Check sheet for the drawn part. Datum: minimum x, y, z corner. Units: mm. A direction names the side the tool comes from. Round coordinates to 2 decimals unless told otherwise and drop trailing zeros. Loops run counter-clockwise (first coordinate to the right, second up) from the corner with the lowest first, then second, coordinate; pieces in that order, holes last.
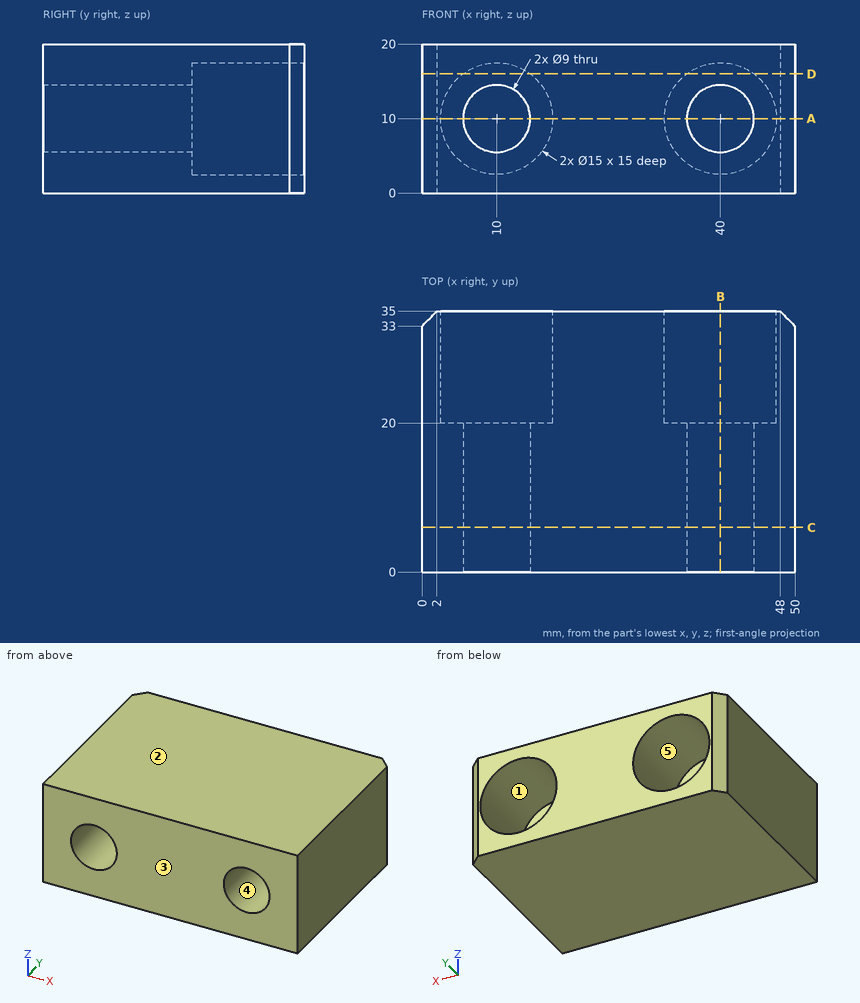
1. Release check for a two-part mould opening along Z. For the marked faces 1, 2 and 3 record: released by +Z, released by -Z, zero draft, split by the parting line, or undercut.
2. Section check D-D (z = 16). Enter the section's corners in (x, y).
3. Section check A-A (z = 10). Enter the section's corners in (x, y).
4. Scan lines: L1, parallel to Z at x = 10, y = 27; L2, parallel to X at y = 27, z = 7; L3, parallel to X at y = 18.5, z = 6.5. Record each from-to range of solid material in increasing order.
5. Gauge pin test, flat ends, axial feed: P1, Ø7.5, axis at x = 39.5, z = 13.5, coming from the +Y side; P2, Ø8, axis at x = 40, z = 10, coming from the -Y side. Record the tip position at first contact, or that the pin passes through.
6. Tool access check on the marked faces 4 and 5. Record the directions out of +Z, -Z, +X, -X, +Y, -Y that give a thin tool (end or side, any length) a straight path to the whole face; none if there is none.
7. Section check B-B (x = 40). Enter the section's corners in (y, z), then the cut area to 3 significant figures.
8. Section check C-C (y = 6). Enter the section's corners in (x, z), then the cut area to 3 significant figures.
Taken from the geometry:
1. face 1: undercut
1. face 2: released by +Z
1. face 3: zero draft
2. outline: (0, 0) - (50, 0) - (50, 33) - (48, 35) - (44.5, 35) - (44.5, 20) - (35.5, 20) - (35.5, 35) - (14.5, 35) - (14.5, 20) - (5.5, 20) - (5.5, 35) - (2, 35) - (0, 33) - close
3. outline: (0, 0) - (5.5, 0) - (5.5, 20) - (2.5, 20) - (2.5, 35) - (2, 35) - (0, 33) - close; (14.5, 0) - (35.5, 0) - (35.5, 20) - (32.5, 20) - (32.5, 35) - (17.5, 35) - (17.5, 20) - (14.5, 20) - close; (44.5, 0) - (50, 0) - (50, 33) - (48, 35) - (47.5, 35) - (47.5, 20) - (44.5, 20) - close
4. L1: z = 0 to 2.5, 17.5 to 20
4. L2: x = 0 to 3.13, 16.87 to 33.13, 46.87 to 50
4. L3: x = 0 to 7.17, 12.83 to 37.17, 42.83 to 50
5. P1: stops at y = 20
5. P2: passes through
6. face 4: +Y, -Y
6. face 5: +Y
7. outline: (0, 0) - (35, 0) - (35, 2.5) - (20, 2.5) - (20, 5.5) - (0, 5.5) - close; (0, 14.5) - (20, 14.5) - (20, 17.5) - (35, 17.5) - (35, 20) - (0, 20) - close
7. area: 295 mm2
8. outline: (0, 0) - (50, 0) - (50, 20) - (0, 20) - close; hole circle Ø9 at (10, 10); hole circle Ø9 at (40, 10)
8. area: 873 mm2
